Work out the finished part from the listing and answer in its coordinate system (mm). A direction names the side the tool comes from. Coordinates: 2 decimals unless noted, no trailing zeros. Order: outer loops, then holes, each group sorted by start corner. A loop starts at its lowest first (then second) coordinate and runs counter-clockwise, first axis right, second up. Notation, with made-up numbers: M 76,-4.75 L 91,-4.75 A26 ccw 91,33.25 Z; hole C -20.75,15.5 d4. An arc over 180 degrees is marked long. Write item = value, one per line. Start each with the question number.
Q1. Find section C-C on y = 132.5. Give the vertices of the cut face in (x, z), and give its area (3 significant figures).
Q2. Each of these flat-tipped pins is pushed along its axis until it touches: P1, Ø10, axis at y = -23.5, z = -12, coming from the +X side; P2, Ø6, axis at y = -62.5, z = 20.5, coming from the -X side; P3, Ø10, axis at x = -6.5, y = -11, coming from the +Z side. Where does it stop, or does it pass through?
Q3. A tool of negligible diameter and unlimited length cuts with its end or side. For faces 1 (the cylindrical face through (-10.648, 112.395, -13.887)), 2 (the flat face through (0, -105, 0)), from which of +Z, -Z, +X, -X, +Y, -Y can it reach the whole face along a straight path? Write none if from no direction.
Q4. Straight lines are drawn through the part: line 1 along Y through (x, z) = (29.5, 1); line 2 along Y through (x, z) = (2, -17); line 3 along X through (y, z) = (-10.5, 25). For each, find the intervals that lie inside material, in ascending order.
Q5. Find section A-A on x = 0. Give the vertices of the cut face in (y, z).
Q6. Find section B-B on y = 56. Give the vertices of the cut face in (x, z), and give its area (3 significant figures).
```python
from build123d import *

# Parameters (mm, degrees)
SKETCH_1_R      = 37
EXTRUDE_1_DEPTH = 105
SKETCH_2_R      = 17.5
EXTRUDE_2_DEPTH = 15
SKETCH_3_R      = 12.5
EXTRUDE_3_DEPTH = 75
SKETCH_4_R      = 10
EXTRUDE_4_DEPTH = 20
SKETCH_5_R      = 8
EXTRUDE_5_DEPTH = 33
FILLET_1_R      = 3


with BuildPart() as part:
    # 草图1 → 凸台-拉伸1 (new, symmetric)
    with BuildSketch(Plane(origin=(0, 0, 0), x_dir=(1, 0, 0), z_dir=(0, 1, 0))):
        with Locations(Location((0, 0, 0), (0, 0, 270))):
            Circle(SKETCH_1_R)
    extrude(amount=EXTRUDE_1_DEPTH, both=True)

    # 草图2 → 凸台-拉伸2 (add)
    with BuildSketch(Plane(origin=(0, 105, 0), x_dir=(1, 0, 0), z_dir=(0, 1, 0))):
        with Locations(Location((0, 0, 0), (0, 0, 270))):
            Circle(SKETCH_2_R)
    extrude(amount=EXTRUDE_2_DEPTH)

    # 草图3 → 凸台-拉伸3 (add)
    with BuildSketch(Plane(origin=(0, 120, 0), x_dir=(1, 0, 0), z_dir=(0, 1, 0))):
        with Locations(Location((0, 0, 0), (0, 0, 270))):
            Circle(SKETCH_3_R)
    extrude(amount=EXTRUDE_3_DEPTH)

    # 草图4 → 凸台-拉伸4 (add)
    with BuildSketch(Plane(origin=(0, 195, 0), x_dir=(1, 0, 0), z_dir=(0, 1, 0))):
        with Locations(Location((0, 0, 0), (0, 0, 270))):
            Circle(SKETCH_4_R)
    extrude(amount=EXTRUDE_4_DEPTH)

    # 草图5 → 凸台-拉伸5 (add)
    with BuildSketch(Plane(origin=(0, 215, 0), x_dir=(1, 0, 0), z_dir=(0, 1, 0))):
        with Locations(Location((0, 0, 0), (0, 0, 270))):
            Circle(SKETCH_5_R)
    extrude(amount=EXTRUDE_5_DEPTH)

    # 圆角1
    fillet_1_edges = [part.edges().sort_by_distance(p)[0] for p in [
        (0, -105, -37),
        (0, 105, -37),
    ]]
    fillet(fillet_1_edges, radius=FILLET_1_R)


solid = part.part
```
Findings below:
q1.outline = C 0,0 d25
q1.area = 491 mm^2
q2.P1 = 36.33
q2.P2 = -32.6
q2.P3 = 36.97
q3.face_1 = +Y
q3.face_2 = +Z, -Z, +X, -X, -Y
q4.line_1 = -105 to 105
q4.line_2 = -105 to 120
q4.line_3 = -27.28 to 27.28
q5.outline = M -105,-34 A3 ccw -102,-37 L 102,-37 A3 ccw 105,-34 L 105,-17.5 L 120,-17.5 L 120,-12.5 L 195,-12.5 L 195,-10 L 215,-10 L 215,-8 L 248,-8 L 248,8 L 215,8 L 215,10 L 195,10 L 195,12.5 L 120,12.5 L 120,17.5 L 105,17.5 L 105,34 A3 ccw 102,37 L -102,37 A3 ccw -105,34 Z
q6.outline = C 0,0 d74
q6.area = 4,300 mm^2
